```python
from build123d import *

# Parameters (mm, degrees)
SKETCH1_W           = 90
SKETCH1_H           = 32
BOSS_EXTRUDE1_DEPTH = 6
SKETCH2_R           = 5.5
CUT_EXTRUDE1_DEPTH  = 6
LPATTERN1_COUNT     = 2
LPATTERN1_PITCH     = 60


with BuildPart() as part:
    # Sketch1 → Boss-Extrude1 (new body)
    with BuildSketch(Plane.XY):
        with Locations((45, -16)):
            Rectangle(SKETCH1_W, SKETCH1_H)
    extrude(amount=BOSS_EXTRUDE1_DEPTH)

    # Sketch2 → Cut-Extrude1 (cut)
    with BuildSketch(Plane.XY.offset(6)):
        with Locations((15, -16)):
            Circle(SKETCH2_R)
    cut_extrude1 = extrude(amount=-CUT_EXTRUDE1_DEPTH, mode=Mode.SUBTRACT)

    # LPattern1: Cut-Extrude1 ×2
    with Locations(*[(i * LPATTERN1_PITCH, 0, 0) for i in range(1, LPATTERN1_COUNT)]):
        add(cut_extrude1, mode=Mode.SUBTRACT)


solid = part.part
```
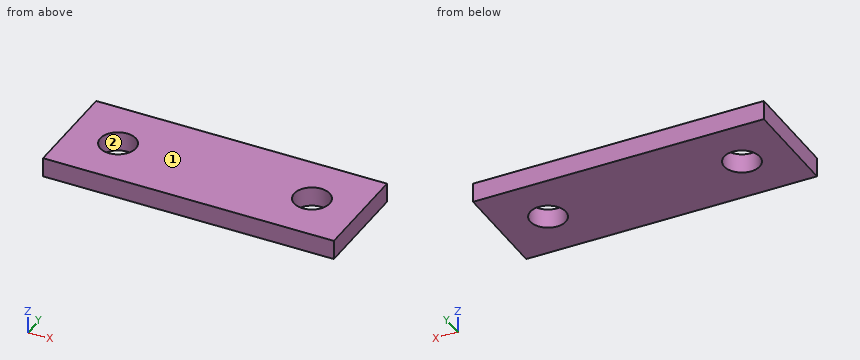
Build history of the part. All positions in model axes, mm. Face numbers are marked on the shaded views. Round coordinates to 2 decimals unless told otherwise and drop trailing zeros. Write each loop counter-clockwise with the first axis right and the second up, starting at its lowest first coordinate (ties: lowest second). Pieces come first, ordered by that corner, then holes.
1) Band-saw the part on A-A, the plane x = 15. List the corners of the cut face in (y, z), and give its area (3 significant figures).
2) Drill centre lines: probe 1 along X at (y, z) = (-11, 4.5); probe 2 along X at (y, z) = (-15, 2.3); probe 3 along Y at (x, z) = (15, 2.95). Where is each one in solid material? Low to high.
3) Band-saw the part on C-C, the plane z = 4.5. List the corners of the cut face in (x, y).
4) Band-saw the part on D-D, the plane y = -20.5. List the corners of the cut face in (x, z), and give its area (3 significant figures).
5) Mould opens along X. For the marked faces 1 and 2 say: +X half, -X half, draft (parallel to the pull), parting line (faces both ways), or undercut.
6) Band-saw the part on B-B, the plane y = -16. List the corners of the cut face in (x, z).
Ans:
1. outline: (-32, 0) - (-21.5, 0) - (-21.5, 6) - (-32, 6) - close; (-10.5, 0) - (0, 0) - (0, 6) - (-10.5, 6) - close
1. area: 126 mm2
2. probe 1: x = 0 to 12.71, 17.29 to 72.71, 77.29 to 90
2. probe 2: x = 0 to 9.59, 20.41 to 69.59, 80.41 to 90
2. probe 3: y = -32 to -21.5, -10.5 to 0
3. outline: (0, -32) - (90, -32) - (90, 0) - (0, 0) - close; hole circle Ø11 at (15, -16); hole circle Ø11 at (75, -16)
4. outline: (0, 0) - (11.84, 0) - (11.84, 6) - (0, 6) - close; (18.16, 0) - (71.84, 0) - (71.84, 6) - (18.16, 6) - close; (78.16, 0) - (90, 0) - (90, 6) - (78.16, 6) - close
4. area: 464 mm2
5. face 1: draft
5. face 2: undercut
6. outline: (0, 0) - (9.5, 0) - (9.5, 6) - (0, 6) - close; (20.5, 0) - (69.5, 0) - (69.5, 6) - (20.5, 6) - close; (80.5, 0) - (90, 0) - (90, 6) - (80.5, 6) - close
